```python
from build123d import *

# Parameters (mm, degrees)
SKETCH1_R           = 65
SKETCH1_R_2         = 15
BOSS_EXTRUDE1_DEPTH = 10
SKETCH2_R           = 5
CUT_EXTRUDE1_DEPTH  = 10
SKETCH3_W           = 40
SKETCH3_H           = 40
BOSS_EXTRUDE2_DEPTH = 50
SKETCH4_W           = 30
SKETCH4_H           = 47
CUT_EXTRUDE2_DEPTH  = 50
SKETCH5_R           = 5
CUT_EXTRUDE3_DEPTH  = 123.678441464


with BuildPart() as part:
    # Sketch1 → Boss-Extrude1 (new body)
    with BuildSketch(Plane(origin=(0, 0, 0), x_dir=(1, 0, 0), z_dir=(0, 1, 0))):
        with Locations(Location((0, 0, 0), (0, 0, 270))):
            Circle(SKETCH1_R)
        with Locations(Location((0, 0, 0), (0, 0, 270))):
            Circle(SKETCH1_R_2, mode=Mode.SUBTRACT)
    extrude(amount=BOSS_EXTRUDE1_DEPTH)

    # Sketch2 → Cut-Extrude1 (cut)
    with BuildSketch(Plane(origin=(0, 10, 0), x_dir=(1, 0, 0), z_dir=(0, 1, 0))):
        with Locations(Location((0, 45, 0), (0, 0, 270))):
            Circle(SKETCH2_R)
        with Locations(Location((45, 0, 0), (0, 0, 270))):
            Circle(SKETCH2_R)
        with Locations(Location((0, -45, 0), (0, 0, 270))):
            Circle(SKETCH2_R)
        with Locations(Location((-45, 0, 0), (0, 0, 270))):
            Circle(SKETCH2_R)
    extrude(amount=-CUT_EXTRUDE1_DEPTH, mode=Mode.SUBTRACT)

    # Sketch3 → Boss-Extrude2 (add)
    with BuildSketch(Plane(origin=(0, 10, 0), x_dir=(1, 0, 0), z_dir=(0, 1, 0))):
        Rectangle(SKETCH3_W, SKETCH3_H)
    extrude(amount=BOSS_EXTRUDE2_DEPTH)

    # Sketch4 → Cut-Extrude2 (cut)
    with BuildSketch(Plane(origin=(20, 0, 0), x_dir=(0, 0, -1), z_dir=(1, 0, 0))):
        with Locations((0, 36.5)):
            Rectangle(SKETCH4_W, SKETCH4_H)
    extrude(amount=-CUT_EXTRUDE2_DEPTH, mode=Mode.SUBTRACT)

    # Sketch5 → Cut-Extrude3 (cut, through all)
    with BuildSketch(Plane.XY.offset(20)):
        with Locations((0, 46.469084147)):
            Circle(SKETCH5_R)
    extrude(amount=-CUT_EXTRUDE3_DEPTH, mode=Mode.SUBTRACT)


solid = part.part
```
Read the model definition and answer for the solid it produces. Units are mm, in the model's axes. A direction names the side the tool comes from. Round coordinates to 2 decimals unless told otherwise and drop trailing zeros. Write each loop counter-clockwise with the first axis right and the second up, starting at its lowest first coordinate (ties: lowest second). Pieces come first, ordered by that corner, then holes. Notation, with made-up numbers: M -5.5,38 L 12.5,38 A23 ccw 12.5,54 Z; hole C 9.5,-13 d6. An arc over 180 degrees is marked long. One line per item, written item: value.
Q1. Find section C-C on y = 37.5. Write down the section's boundary in (x, z).
Data:
outline: M -20,-20 L 20,-20 L 20,-15 L -20,-15 Z; M -20,15 L 20,15 L 20,20 L -20,20 Z
Q2. Find section B-B on x = 0. Count the separate pieces of the cut face and the enclosed holes in it, plus the area to 3 significant figures.
Data:
separate pieces: 5
enclosed holes: 0
area: 1,290 mm2
Q3. Find section D-D on x = -42. Write down the section's boundary in (y, z), plus the area to 3 significant figures.
Data:
outline: M 0,-49.61 L 10,-49.61 L 10,-4 L 0,-4 Z; M 0,4 L 10,4 L 10,49.61 L 0,49.61 Z
area: 912 mm2
Q4. Straight lines are drawn through the part: line 1 (X direction, y = 6.25, z = 0); line 2 (Z direction, x = -3.5, y = 42.5); line 3 (Y direction, x = 0, z = 16.75). For each, find the intervals that lie inside material, in ascending order. Write a range as [from, to].
Data:
line 1: [-65, -50], [-40, -15], [15, 40], [50, 65]
line 2: [-20, -15], [15, 20]
line 3: [0, 41.47], [51.47, 60]
Q5. For a pull along X with two mould halves and no side action, classify faces 1 (the flat face through (20, 29, 16)), 2 (the cylindrical face through (49.957, 5.07, -0.651)), 3 (the cylindrical face through (19.52, 4.93, 62)) as +X half, -X half, draft (parallel to the pull), parting line (faces both ways), or undercut.
Data:
face 1: +X half
face 2: undercut
face 3: parting line
Q6. Which of the six approach directions +Z, -Z, +X, -X, +Y, -Y give full straight-line access (tool end or side, diameter ignored) to faces 4 (the flat face through (1, 10, 28)), 5 (the flat face through (0, 36, -15)), 6 (the cylindrical face through (0.66, 4.93, -14.985)), 7 (the flat face through (-20, 29, 16)), 8 (the flat face through (0, 35, 20))?
Data:
face 4: +Y
face 5: +X, -X, +Y
face 6: -Y
face 7: +Z, -Z, -X, +Y
face 8: +Z, +X, -X, +Y
Q7. Flat-ended cylindrical pins translate along their axes: pin 1 Ø9 at (x, z) = (0, 45) entering from +Y; pin 2 Ø24 at (x, z) = (0, 0) entering from -Y; pin 3 Ø13 at (x, z) = (-45, 0) entering from +Y; pin 4 Ø16 at (x, y) = (0, 46.47) entering from +Z. Find the tip coordinate at first contact, or state that the pin passes through.
Data:
pin 1: through
pin 2: y = 10
pin 3: y = 10
pin 4: z = 20
Q8. Find section A-A on z = 0. Write down the section's boundary in (x, y), plus the area to 3 significant figures.
Data:
outline: M -65,0 L -50,0 L -50,10 L -65,10 Z; M -40,0 L -15,0 L -15,10 L 15,10 L 15,0 L 40,0 L 40,10 L 20,10 L 20,13 L -20,13 L -20,10 L -40,10 Z; M 50,0 L 65,0 L 65,10 L 50,10 Z
area: 920 mm2
